from build123d import *

# Parameters (mm, degrees)
BOSS_EXTRUDE1_DEPTH     = 2
BOSS_EXTRUDE2_START     = 178
BOSS_EXTRUDE2_DEPTH     = 178
CUT_EXTRUDE1_DEPTH      = 415.686930105
CUT_EXTRUDE1_DEPTH_BACK = 415.686930105
SKETCH3_R               = 6
SKETCH4_R               = 5
CUT_EXTRUDE2_DEPTH      = 693.095730373
SKETCH5_R               = 6
BOSS_EXTRUDE3_DEPTH     = 2


with BuildPart() as part:
    # Sketch1 → Boss-Extrude1 (new body)
    with BuildSketch(Plane.XY):
        with BuildLine():
            Line((-335, -167.5), (-335, 157.5))
            ThreePointArc((-335, 157.5), (-332.071067812, 164.571067812), (-325, 167.5))
            Line((-325, 167.5), (325, 167.5))
            ThreePointArc((325, 167.5), (332.071067812, 164.571067812), (335, 157.5))
            Line((335, 157.5), (335, -167.5))
            Line((335, -167.5), (310, -167.5))
            Line((310, -167.5), (310, 132.5))
            ThreePointArc((310, 132.5), (307.071067812, 139.571067812), (300, 142.5))
            Line((300, 142.5), (-300, 142.5))
            ThreePointArc((-300, 142.5), (-307.071067812, 139.571067812), (-310, 132.5))
            Line((-310, 132.5), (-310, -167.5))
            Line((-310, -167.5), (-335, -167.5))
        make_face()
    extrude(amount=BOSS_EXTRUDE1_DEPTH)

    # Sketch2 → Boss-Extrude2 (add)
    with BuildSketch(Plane(origin=(0, 0, 0), x_dir=(-1, 0, 0), z_dir=(0, 0, -1)).offset(BOSS_EXTRUDE2_START)):
        with BuildLine():
            Line((310, -167.5), (310, 132.5))
            ThreePointArc((310, 132.5), (307.071067812, 139.571067812), (300, 142.5))
            Line((300, 142.5), (-300, 142.5))
            ThreePointArc((-300, 142.5), (-307.071067812, 139.571067812), (-310, 132.5))
            Line((-310, 132.5), (-310, -167.5))
            Line((-310, -167.5), (-312.5, -167.5))
            Line((-312.5, -167.5), (-312.5, 135))
            ThreePointArc((-312.5, 135), (-309.571067812, 142.071067812), (-302.5, 145))
            Line((-302.5, 145), (302.5, 145))
            ThreePointArc((302.5, 145), (309.571067812, 142.071067812), (312.5, 135))
            Line((312.5, 135), (312.5, -167.5))
            Line((312.5, -167.5), (310, -167.5))
        make_face()
    extrude(amount=-BOSS_EXTRUDE2_DEPTH)

    # Sketch3 → Cut-Extrude1 (cut, two sides: drawn at the far end of the back side and taken through both)
    with BuildSketch(Plane(origin=(0, 0, 0), x_dir=(-1, 0, 0), z_dir=(0, 0, -1)).offset(-CUT_EXTRUDE1_DEPTH_BACK)):
        with Locations((0, 155.5)):
            Circle(SKETCH3_R)
        with Locations((-161.5, 155.5)):
            Circle(SKETCH3_R)
        with Locations((-323, 12.5)):
            Circle(SKETCH3_R)
        with Locations((-323, -107.5)):
            Circle(SKETCH3_R)
        with Locations((-323, 155.5)):
            Circle(SKETCH3_R)
        with Locations((323, 155.5)):
            Circle(SKETCH3_R)
        with Locations((323, -107.5)):
            Circle(SKETCH3_R)
        with Locations((323, 12.5)):
            Circle(SKETCH3_R)
        with Locations((161.5, 155.5)):
            Circle(SKETCH3_R)
    extrude(amount=CUT_EXTRUDE1_DEPTH + CUT_EXTRUDE1_DEPTH_BACK, mode=Mode.SUBTRACT)

    # Sketch4 → Cut-Extrude2 (cut, through all)
    with BuildSketch(Plane(origin=(312.5, 0, 0), x_dir=(0, 0, -1), z_dir=(1, 0, 0))):
        with Locations((88, 82.5)):
            Circle(SKETCH4_R)
        with Locations((88, -17.5)):
            Circle(SKETCH4_R)
        with Locations((88, -117.5)):
            Circle(SKETCH4_R)
    extrude(amount=-CUT_EXTRUDE2_DEPTH, mode=Mode.SUBTRACT)

    # Sketch5 → Boss-Extrude3 (add)
    with BuildSketch(Plane(origin=(0, 0, -178), x_dir=(-1, 0, 0), z_dir=(0, 0, -1))):
        with BuildLine():
            Line((-312.5, -167.5), (-312.5, 135))
            ThreePointArc((-312.5, 135), (-309.571067812, 142.071067812), (-302.5, 145))
            Line((-302.5, 145), (302.5, 145))
            ThreePointArc((302.5, 145), (309.571067812, 142.071067812), (312.5, 135))
            Line((312.5, 135), (312.5, -167.5))
            Line((312.5, -167.5), (335, -167.5))
            Line((335, -167.5), (335, 157.5))
            ThreePointArc((335, 157.5), (332.071067812, 164.571067812), (325, 167.5))
            Line((325, 167.5), (-325, 167.5))
            ThreePointArc((-325, 167.5), (-332.071067812, 164.571067812), (-335, 157.5))
            Line((-335, 157.5), (-335, -167.5))
            Line((-335, -167.5), (-312.5, -167.5))
        make_face()
        with Locations((-323, -107.5)):
            Circle(SKETCH5_R, mode=Mode.SUBTRACT)
        with Locations((-323, 12.5)):
            Circle(SKETCH5_R, mode=Mode.SUBTRACT)
        with Locations((-161.5, 155.5)):
            Circle(SKETCH5_R, mode=Mode.SUBTRACT)
        with Locations((0, 155.5)):
            Circle(SKETCH5_R, mode=Mode.SUBTRACT)
        with Locations((161.5, 155.5)):
            Circle(SKETCH5_R, mode=Mode.SUBTRACT)
        with Locations((323, 12.5)):
            Circle(SKETCH5_R, mode=Mode.SUBTRACT)
        with Locations((323, -107.5)):
            Circle(SKETCH5_R, mode=Mode.SUBTRACT)
        with Locations((323, 155.5)):
            Circle(SKETCH5_R, mode=Mode.SUBTRACT)
        with Locations((-323, 155.5)):
            Circle(SKETCH5_R, mode=Mode.SUBTRACT)
    extrude(amount=-BOSS_EXTRUDE3_DEPTH)


solid = part.part
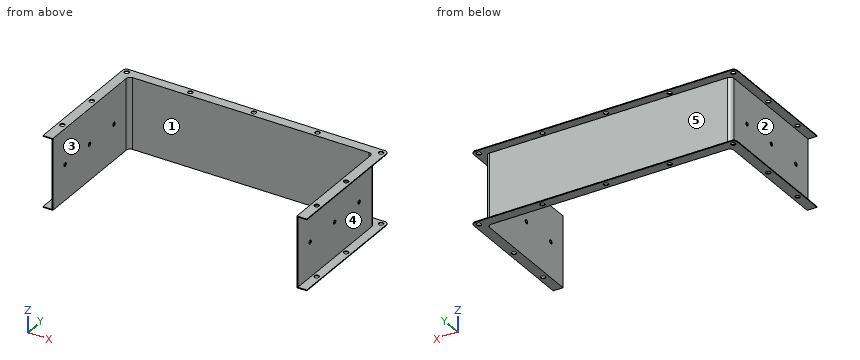
Model file for the job. Use its own axes, mm. Face numbers are marked on the shaded views. A direction names the side the tool comes from. Give positions to 0.01 mm unless a question says otherwise; leave off trailing zeros. Order: outer loops, then holes, each group sorted by start corner. A loop starts at its lowest first (then second) coordinate and runs counter-clockwise, first axis right, second up. Notation, with made-up numbers: M -35.5,35.25 L -17.5,35.25 A19 cw -17.5,72.25 Z; hole C 81,33 d10. An arc over 180 degrees is marked long. Put each result on its own line as item: value. Start each with the question number.
(1) Pull direction Z, two halves, no side cores. Call the marked faces 1 and 2: released by +Z, released by -Z, zero draft, split by the parting line, or undercut.
(2) Drill centre lines: L1, parallel to Y at x = 323, z = 1; L2, parallel to X at y = 155.5, z = 1.1; L3, parallel to X at y = 11, z = -60. Where is each one in solid material? Low to high. Write a range as [from, to].
(3) Band-saw the part on B-B on x = 51. Give the cut face in (y, z).
(4) Tool access for the marked faces 3, 4 and 5: list every direction of +Z, -Z, +X, -X, +Y, -Y with a clear straight run to the whole face (end or side of a thin tool).
(5) Band-saw the part on C-C on z = -75. Give the cut face in (x, y), then the cut area to 3 significant figures.
(6) Pin check, flat tips, straight feed: pin 1 Ø8 at (x, z) = (-248.5, -79.5) entering from -Y; pin 2 Ø10 at (x, z) = (134, -117) entering from +Y; pin 3 Ø12 at (y, z) = (90.5, -83) entering from -X. Stop position of each tip, or through.
(7) Band-saw the part on A-A on y = -49. Give the cut face in (x, z), then the cut area to 3 significant figures.
Results below:
1. face 1: zero draft
1. face 2: undercut
2. L1: y = [-167.5, -113.5], [-101.5, 6.5], [18.5, 149.5], [161.5, 167.5]
2. L2: x = [-335, -329], [-317, -167.5], [-155.5, -6], [6, 155.5], [167.5, 317], [329, 335]
2. L3: x = [-312.5, -310], [310, 312.5]
3. outline: M 142.5,-178 L 167.5,-178 L 167.5,-176 L 145,-176 L 145,0 L 167.5,0 L 167.5,2 L 142.5,2 Z
4. face 3: +Z, -Z, -Y
4. face 4: +X, +Y, -Y
4. face 5: +X, -X, +Y
5. outline: M -312.5,-167.5 L -310,-167.5 L -310,132.5 A10 cw -300,142.5 L 300,142.5 A10 cw 310,132.5 L 310,-167.5 L 312.5,-167.5 L 312.5,135 A10 ccw 302.5,145 L -302.5,145 A10 ccw -312.5,135 Z
5. area: 3,110 mm2
6. pin 1: stops at y = 142.5
6. pin 2: stops at y = 145
6. pin 3: stops at x = -312.5
7. outline: M -335,-178 L -310,-178 L -310,2 L -335,2 L -335,0 L -312.5,0 L -312.5,-176 L -335,-176 Z; M 310,-178 L 335,-178 L 335,-176 L 312.5,-176 L 312.5,0 L 335,0 L 335,2 L 310,2 Z
7. area: 1,080 mm2
